```python
from build123d import *

# Parameters (mm, degrees)
SKETCH1_W           = 120
SKETCH1_H           = 200
BOSS_EXTRUDE1_DEPTH = 40
FILLET1_R           = 10


with BuildPart() as part:
    # Sketch1 → Boss-Extrude1 (new body)
    with BuildSketch(Plane.XY):
        with BuildLine():
            Line((1420, 840), (1295, 840))
            ThreePointArc((1295, 840), (1287.928932188, 837.071067812), (1285, 830))
            Line((1285, 830), (1285, 690))
            ThreePointArc((1285, 690), (1287.928932188, 682.928932188), (1295, 680))
            Line((1295, 680), (1420, 680))
            Line((1420, 680), (1420, 580))
            Line((1420, 580), (1295, 580))
            ThreePointArc((1295, 580), (1287.928932188, 577.071067812), (1285, 570))
            Line((1285, 570), (1285, 430))
            ThreePointArc((1285, 430), (1287.928932188, 422.928932188), (1295, 420))
            Line((1295, 420), (1420, 420))
            Line((1420, 420), (1420, 320))
            Line((1420, 320), (1295, 320))
            ThreePointArc((1295, 320), (1287.928932188, 317.071067812), (1285, 310))
            Line((1285, 310), (1285, 170))
            ThreePointArc((1285, 170), (1287.928932188, 162.928932188), (1295, 160))
            Line((1295, 160), (1420, 160))
            Line((1420, 160), (1420, 0))
            Line((1420, 0), (0, 0))
            Line((0, 0), (0, 1000))
            Line((0, 1000), (1420, 1000))
            Line((1420, 1000), (1420, 840))
        make_face()
        with Locations((237, 500)):
            Rectangle(SKETCH1_W, SKETCH1_H, mode=Mode.SUBTRACT)
    extrude(amount=BOSS_EXTRUDE1_DEPTH)

    # Fillet1
    fillet1_edges = [part.edges().sort_by_distance(p)[0] for p in [
        (0, 1000, 20),
        (0, 0, 20),
    ]]
    fillet(fillet1_edges, radius=FILLET1_R)


solid = part.part
```
Build history of the part. All positions in model axes, mm. A direction names the side the tool comes from. Round coordinates to 2 decimals unless told otherwise and drop trailing zeros. Loops run counter-clockwise (first coordinate to the right, second up) from the corner with the lowest first, then second, coordinate; pieces in that order, holes last.
Item 1: Pin check, flat tips, straight feed: P1, Ø20, axis at y = 496.5, z = 12, coming from the +X side; P2, Ø10, axis at x = 1048, y = 422, coming from the -Z side. Stop position of each tip, or through.
Item 2: Saw through at A-A (x = 221). List the corners of the cut face in (y, z), then the cut area to 3 significant figures.
Item 3: Two-plate mould, pull along Y, no slides. Class faces 4 (the face through (1358, 580, 20)), 5 (the face through (705, 1000, 20)), 6 (the face through (1420, 81, 20)): released by +Y, released by -Y, zero draft, split by the parting line, or undercut.
Item 4: Saw through at C-C (y = 746). List the corners of the cut face in (x, z), then the cut area to 3 significant figures.
Item 5: Which spindle directions (+Z, -Z, +X, -X, +Y, -Y) get a long thin tool onto all of the face, cutting with end or side? Do faces 1 (the face through (1285, 501, 20)), 2 (the face through (236, 400, 20)), 3 (the face through (0, 493, 20)). Say none if no direction does.
Item 6: Saw through at B-B (z = 20). List the corners of the cut face in (x, y).
Item 7: Drill centre lines: line 1 along X through (y, z) = (506, 11); line 2 along X through (y, z) = (705, 38). Where is each one in solid material? Low to high.
Worked answers:
1. P1: stops at x = 1285
1. P2: stops at z = 0
2. outline: (0, 0) - (400, 0) - (400, 40) - (0, 40) - close; (600, 0) - (1000, 0) - (1000, 40) - (600, 40) - close
2. area: 32,000 mm2
3. face 4: undercut
3. face 5: released by +Y
3. face 6: zero draft
4. outline: (0, 0) - (1285, 0) - (1285, 40) - (0, 40) - close
4. area: 51,400 mm2
5. face 1: +Z, -Z, +X
5. face 2: +Z, -Z
5. face 3: +Z, -Z, -X, +Y, -Y
6. outline: (0, 10) arc R10 ccw to (10, 0) - (1420, 0) - (1420, 160) - (1295, 160) arc R10 cw to (1285, 170) - (1285, 310) arc R10 cw to (1295, 320) - (1420, 320) - (1420, 420) - (1295, 420) arc R10 cw to (1285, 430) - (1285, 570) arc R10 cw to (1295, 580) - (1420, 580) - (1420, 680) - (1295, 680) arc R10 cw to (1285, 690) - (1285, 830) arc R10 cw to (1295, 840) - (1420, 840) - (1420, 1000) - (10, 1000) arc R10 ccw to (0, 990) - close; hole (177, 400) - (297, 400) - (297, 600) - (177, 600) - close
7. line 1: x = 0 to 177, 297 to 1285
7. line 2: x = 0 to 1285
